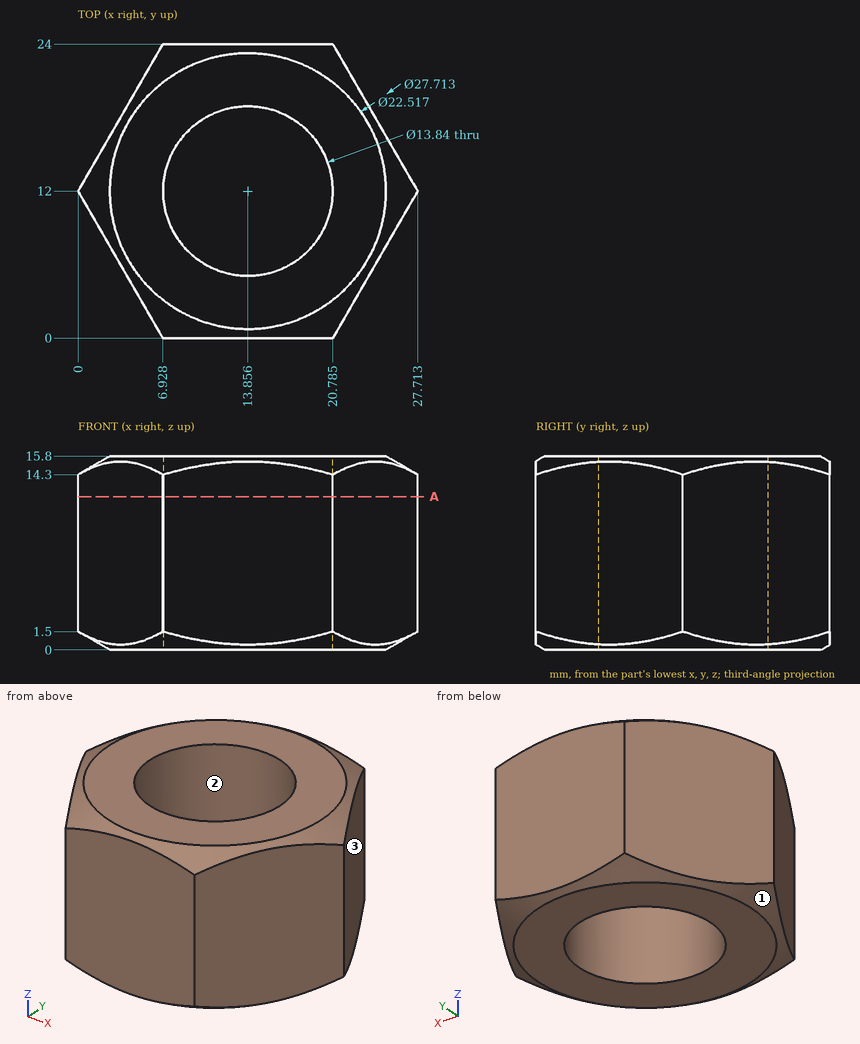
Geometry: see drawing. Coordinates: mm, zero at the bounding-box minimum. Round coordinates to 2 decimals unless told otherwise and drop trailing zeros. Write each loop counter-clockwise with the first axis right and the second up, starting at its lowest first coordinate (ties: lowest second). Pieces come first, ordered by that corner, then holes. Notation, with made-up numbers: M -6,47.5 L 30,47.5 A14 ccw 30,51.5 Z; hole C 57,16.25 d2. An arc over 180 degrees is marked long. Answer in a Markdown table with one row per item. Add a question column.
(1) Draft query along Y for the marked faces 1, 2 and 3. Return one class per face: pulls with the +Y half, pulls with the -Y half, needs draft (parallel to the pull), parting line crosses it, or undercut.
(2) Cut plane A-A, the plane z = 12.5. Return the cut outline in (x, y) (1 decimal), then the cut area to 3 significant figures.
(3) Contact query for flat-ended pins moving along their axis: pin 1 (2 mm diameter, centred on y = 7, z = 12.5, fed in from +X); pin 2 (3 mm diameter, centred on y = 3, z = 10.5, fed in from -X); pin 3 (2 mm diameter, centred on y = 14, z = 13.5, fed in from +X) (1 decimal). Output: stop coordinate, or through.
(4) Ray query, L1, parallel to Y at x = 15.25, z = 8; L2, parallel to Y at x = 6.5, z = 10.75 (1 decimal); L3, parallel to Y at x = 8.5, z = 5. Return the intervals inside material, ascending.
Established:
| question | item | result |
|---|---|---|
| 1 | face 1 | parting line crosses it |
| 1 | face 2 | undercut |
| 1 | face 3 | pulls with the +Y half |
| 2 | outline | M 0,12 L 6.9,0 L 20.8,0 L 27.7,12 L 20.8,24 L 6.9,24 Z; hole C 13.9,12 d13.8 |
| 2 | area | 348 mm² |
| 3 | pin 1 | x = 25.4 |
| 3 | pin 2 | x = 4.33 |
| 3 | pin 3 | x = 27.1 |
| 4 | L1 | 0 to 5.22, 18.78 to 24 |
| 4 | L2 | 0.7 to 23.3 |
| 4 | L3 | 0 to 7.62, 16.38 to 24 |
